Geometry check sheet. Reference: the model listing, model coordinates, mm. A direction names the side the tool comes from. Coordinates: 2 decimals unless noted, no trailing zeros. Loops run counter-clockwise (first coordinate to the right, second up) from the corner with the lowest first, then second, coordinate; pieces in that order, holes last.
from build123d import *
from build123d.topology import SkipClean

# Parameters (mm, degrees)
BASE_BLOCK_SKETCH_W             = 130
BASE_BLOCK_SKETCH_H             = 90
BASE_BLOCK_40_DEPTH             = 40
SIDE_POCKET_A_25_DEPTH          = 25
SIDE_POCKET_B_25_DEPTH          = 25
UPPER_BOSS_50_DEPTH             = 50
WEB_BOSS_10_DEPTH               = 10
WEB_NOTCH_A_10_DEPTH            = 10
WEB_NOTCH_B_10_DEPTH            = 10
SLOT_CUT_A_60_DEPTH             = 60
SLOT_START                      = -60
SLOT_CUT_B_60_DEPTH             = 60
SLOT_CUT_C_60_DEPTH             = 60
SPOT_FACE_A_SKETCH_R            = 15
SPOT_FACE_A_30X5_DEPTH          = 5
SPOT_FACE_B_SKETCH_R            = 15
SPOT_FACE_B_30X5_DEPTH          = 5
BEARING_CRADLE_50_THROUGH_DEPTH = 130


with BuildPart() as part:
    # Base Block Sketch → Base Block 40 (new body)
    with BuildSketch(Plane.XY):
        with Locations((65, 45)):
            Rectangle(BASE_BLOCK_SKETCH_W, BASE_BLOCK_SKETCH_H)
    extrude(amount=BASE_BLOCK_40_DEPTH)

    # Side Pocket A Sketch → Side Pocket A 25 (cut)
    with BuildSketch(Plane.XZ):
        Polygon((65, 40), (40, 40), (40, 25), (90, 25), (90, 40), align=None)
    extrude(amount=-SIDE_POCKET_A_25_DEPTH, mode=Mode.SUBTRACT)

    # Side Pocket B Sketch → Side Pocket B 25 (cut)
    with BuildSketch(Plane(origin=(0, 90, 0), x_dir=(1, 0, 0), z_dir=(0, 1, 0))):
        Polygon((65, -40), (90, -40), (90, -25), (40, -25), (40, -40), align=None)
    extrude(amount=-SIDE_POCKET_B_25_DEPTH, mode=Mode.SUBTRACT)

    # Upper Boss Sketch → Upper Boss 50 (add)
    with BuildSketch(Plane.XZ.offset(-25)):
        Polygon((65, 100), (105, 100), (130, 40), (0, 40), (25, 100), align=None)
    extrude(amount=-UPPER_BOSS_50_DEPTH)

    # Web Boss Sketch → Web Boss 10 (add)
    with BuildSketch(Plane.XZ.offset(-25)):
        Polygon((0, 40), (25, 100), (105, 100), (130, 40), (90, 40), (40, 40), align=None)
    extrude(amount=WEB_BOSS_10_DEPTH)

    # Web Notch A Sketch → Web Notch A 10 (cut)
    with BuildSketch(Plane.XZ.offset(-15)):
        with BuildLine():
            Line((90, 100), (40, 100))
            ThreePointArc((40, 100), (65, 75), (90, 100))
        make_face()
        with BuildLine():
            ThreePointArc((40, 100), (65, 75), (90, 100))
            Line((90, 100), (90, 40))
            Line((90, 40), (40, 40))
            Line((40, 40), (40, 100))
        make_face()
    extrude(amount=-WEB_NOTCH_A_10_DEPTH, mode=Mode.SUBTRACT)

    # Web Notch B Sketch → Web Notch B 10 (cut)
    with BuildSketch(Plane(origin=(0, 75, 0), x_dir=(1, 0, 0), z_dir=(0, 1, 0))):
        with BuildLine():
            ThreePointArc((90, -100), (65, -75), (40, -100))
            Line((40, -100), (40, -40))
            Line((40, -40), (90, -40))
            Line((90, -40), (90, -100))
        make_face()
        with BuildLine():
            ThreePointArc((90, -100), (65, -75), (40, -100))
            Line((40, -100), (90, -100))
        make_face()
    extrude(amount=-WEB_NOTCH_B_10_DEPTH, mode=Mode.SUBTRACT)

    # Slot Cut A Sketch → Slot Cut A 60 (cut)
    with BuildSketch(Plane.XZ.offset(-25)):
        with BuildLine():
            Line((35, 100), (95, 100))
            ThreePointArc((95, 100), (65, 70), (35, 100))
        make_face()
    extrude(amount=-SLOT_CUT_A_60_DEPTH, mode=Mode.SUBTRACT)

    # Slot Cut B Sketch → Slot Cut B 60 (cut)
    with SkipClean():  # the faces are left unmerged after this step: merging them gives an invalid solid
        with BuildSketch(Plane(origin=(0, 25, 0), x_dir=(1, 0, 0), z_dir=(0, 1, 0)).offset(SLOT_START)):
            with BuildLine():
                Line((40, -100), (40, -83.416876048))
                ThreePointArc((40, -83.416876048), (36.277186767, -91.339745962), (35, -100))
                Line((35, -100), (40, -100))
            make_face()
            with BuildLine():
                Line((90, -100), (90, -83.416876048))
                ThreePointArc((90, -83.416876048), (93.722813233, -91.339745962), (95, -100))
                Line((95, -100), (90, -100))
            make_face()
        extrude(amount=SLOT_CUT_B_60_DEPTH, mode=Mode.SUBTRACT)

    # Slot Cut C Sketch → Slot Cut C 60 (cut)
    with SkipClean():  # the faces are left unmerged after this step: merging them gives an invalid solid
        with BuildSketch(Plane.XY.offset(100)):
            Polygon((25, 55), (105, 55), (130, 55), (130, 35), (0, 35), (0, 55), align=None)
        extrude(amount=-SLOT_CUT_C_60_DEPTH, mode=Mode.SUBTRACT)

    # Spot Face A Sketch → Spot Face A Ø30x5 (cut)
    with SkipClean():  # the faces are left unmerged after this step: merging them gives an invalid solid
        with BuildSketch(Plane.XZ.offset(-25)):
            with Locations(Location((60, 45, 0), (0, 0, 270))):
                Circle(SPOT_FACE_A_SKETCH_R)
        extrude(amount=-SPOT_FACE_A_30X5_DEPTH, mode=Mode.SUBTRACT)

    # Spot Face B Sketch → Spot Face B Ø30x5 (cut)
    with SkipClean():  # the faces are left unmerged after this step: merging them gives an invalid solid
        with BuildSketch(Plane(origin=(0, 65, 0), x_dir=(1, 0, 0), z_dir=(0, 1, 0))):
            with Locations(Location((70, -45, 0), (0, 0, 270))):
                Circle(SPOT_FACE_B_SKETCH_R)
        extrude(amount=-SPOT_FACE_B_30X5_DEPTH, mode=Mode.SUBTRACT)

    # Bearing Cradle Sketch → Bearing Cradle Ø50 Through (cut)
    with SkipClean():  # the faces are left unmerged after this step: merging them gives an invalid solid
        with BuildSketch(Plane(origin=(130, 0, 0), x_dir=(0, 0, -1), z_dir=(1, 0, 0))):
            with BuildLine():
                Line((0, 70), (0, 20))
                ThreePointArc((0, 20), (-25, 45), (0, 70))
            make_face()
        extrude(amount=-BEARING_CRADLE_50_THROUGH_DEPTH, mode=Mode.SUBTRACT)


solid = part.part
(1) Scan lines: L1, parallel to Y at x = 33, z = 40.5; L2, parallel to Y at x = 54, z = 47; L3, parallel to X at y = 62.45, z = 45. Record each from-to range of solid material in increasing order.
Findings:
L1: y = 15 to 35, 55 to 75
L2: y = 30 to 35, 55 to 65
L3: x = 2.08 to 55, 85 to 127.92
(2) Sectioned sample at A-A on x = 11. Record the cut outline in (y, z).
Findings:
outline: (0, 0) - (20, 0) arc R25 cw to (70, 0) - (90, 0) - (90, 40) - (75, 40) - (75, 66.4) - (55, 66.4) - (55, 40) - (35, 40) - (35, 66.4) - (15, 66.4) - (15, 40) - (0, 40) - close
(3) Draft check along Z on faces 1 (the flat face through (65, 65, 60)), 2 (the flat face through (66, 45, 40)), 3 (the cylindrical face through (55.357, 62.535, 41.748)). Enter one of: +Z half, -Z half, draft (parallel to the pull), parting line (faces both ways), or undercut.
Findings:
face 1: draft
face 2: +Z half
face 3: undercut
(4) Gauge pin test, flat ends, axial feed: pin 1 Ø22 at (x, y) = (61.5, 43.5) entering from +Z; pin 2 Ø12.5 at (x, y) = (57, 79) entering from +Z; pin 3 Ø6 at (x, y) = (72.5, 53.5) entering from -Z. Record the tip position at first contact, or that the pin passes through.
Findings:
pin 1: stops at z = 71.89
pin 2: stops at z = 25
pin 3: stops at z = 22.2
(5) Access from +Z, -Z, +X, -X, +Y, -Y to the whole of each face (thin tool, end or side, straight path). Record for faces 4 (the flat face through (66, 55, 64)), 5 (the flat face through (25, 15, 64)), 6 (the flat face through (40, 72, 48)), 7 (the flat face through (110, 83, 40)), 8 (the flat face through (40, 18, 47)).
Findings:
face 4: +Z, +X, -X
face 5: +Z, +X, -X, -Y
face 6: +Z, +Y
face 7: +Z, +X, -X, +Y
face 8: +Z, -Y
(6) Sectioned sample at D-D on x = 33.5. Record the cut outline in (y, z).
Findings:
outline: (0, 0) - (20, 0) arc R25 cw to (70, 0) - (90, 0) - (90, 40) - (75, 40) - (75, 100) - (55, 100) - (55, 40) - (35, 40) - (35, 100) - (15, 100) - (15, 40) - (0, 40) - close
(7) Sectioned sample at C-C on z = 28.5. Record the cut outline in (x, y).
Findings:
outline: (0, 0) - (40, 0) - (40, 25) - (90, 25) - (90, 0) - (130, 0) - (130, 90) - (90, 90) - (90, 65) - (40, 65) - (40, 90) - (0, 90) - close
(8) Sectioned sample at B-B on z = 51. Record the cut outline in (x, y), and give its area (3 significant figures).
Findings:
outline: (4.58, 15) - (40, 15) - (40, 25) - (46.25, 25) - (46.25, 30) - (73.75, 30) - (73.75, 25) - (90, 25) - (90, 15) - (125.42, 15) - (125.42, 35) - (4.58, 35) - close; (4.58, 55) - (125.42, 55) - (125.42, 75) - (90, 75) - (90, 65) - (83.75, 65) - (83.75, 60) - (56.25, 60) - (56.25, 65) - (40, 65) - (40, 75) - (4.58, 75) - close
area: 3,560 mm2
